```python
from build123d import *

# Parameters (mm, degrees)
BRACKET_BODY_DEPTH      = 35
EYE_END_ROUND_RADIUS    = 35
EYE_END_ROUND_LENGTH    = 20
FORK_GAP_CUT_DEPTH      = 106.59356041
FORK_GAP_CUT_DEPTH_BACK = 106.59356041
FORK_SLOT_CUT_DEPTH     = 15
EYE_BORE_30_REACH       = 110.858
EYE_BORE_SKETCH_R       = 15


with BuildPart() as part:
    # Bracket Profile Sketch → Bracket Body (new, symmetric)
    with BuildSketch(Plane.XY):
        with BuildLine():
            Line((40, -20), (0, -20))
            ThreePointArc((0, -20), (-20, 0), (0, 20))
            Line((0, 20), (40, 20))
            Line((40, 20), (40, 30))
            Line((40, 30), (-20, 30))
            Line((-20, 30), (-40, 10))
            Line((-40, 10), (-95, 10))
            Line((-95, 10), (-95, -10))
            Line((-95, -10), (-40, -10))
            Line((-40, -10), (-20, -30))
            Line((-20, -30), (40, -30))
            Line((40, -30), (40, -20))
        make_face()
    extrude(amount=BRACKET_BODY_DEPTH, both=True)

    # Eye End Round: full round fillet: the end face becomes a half cylinder, R = half its width
    eye_end_round_face = Plane((-95, 0, 0), x_dir=(0, -1, 0), z_dir=(-1, 0, 0))  # on the end face: x along it, z out of the body
    eye_end_round_slab = eye_end_round_face.offset(-EYE_END_ROUND_RADIUS / 2) * Box(EYE_END_ROUND_LENGTH, 2 * EYE_END_ROUND_RADIUS, EYE_END_ROUND_RADIUS, mode=Mode.PRIVATE)  # the body's end, R deep
    eye_end_round_round = Plane((-60, 0, 0), x_dir=(-1, 0, 0), z_dir=(0, -1, 0)) * Cylinder(EYE_END_ROUND_RADIUS, EYE_END_ROUND_LENGTH, mode=Mode.PRIVATE)  # its axis R under the face
    add(eye_end_round_slab - eye_end_round_round, mode=Mode.SUBTRACT)

    # Fork Gap Sketch → Fork Gap Cut (cut, two sides: drawn at the far end of the back side and taken through both)
    with BuildSketch(Plane(origin=(0, 0, 0), x_dir=(1, 0, 0), z_dir=(0, 1, 0)).offset(-FORK_GAP_CUT_DEPTH_BACK)):
        with BuildLine():
            Line((40, 10), (25, 10))
            ThreePointArc((25, 10), (15, 0), (25, -10))
            Line((25, -10), (40, -10))
            Line((40, -10), (40, 10))
        make_face()
    extrude(amount=FORK_GAP_CUT_DEPTH + FORK_GAP_CUT_DEPTH_BACK, mode=Mode.SUBTRACT)

    # Fork Slot Sketch → Fork Slot Cut (cut, symmetric)
    with BuildSketch(Plane.XY):
        Polygon((-40, 10), (-30, 10), (-30, 20), align=None)
    fork_slot_cut = extrude(amount=FORK_SLOT_CUT_DEPTH, both=True, mode=Mode.SUBTRACT)

    # Eye Bore Sketch → Eye Bore _30 (cut, up to next)
    with BuildSketch(Plane(origin=(0, 10, 0), x_dir=(1, 0, 0), z_dir=(0, 1, 0)), mode=Mode.PRIVATE) as eye_bore_30_sk1:
        with Locations(Location((-60, 0, 0), (0, 0, 180))):
            Circle(EYE_BORE_SKETCH_R)
    eye_bore_30_tool1 = extrude(eye_bore_30_sk1.sketch, amount=-EYE_BORE_30_REACH, mode=Mode.PRIVATE) & part.part
    add(eye_bore_30_tool1.solids().sort_by_distance((-60, 10, 0))[0], mode=Mode.SUBTRACT)

    # Fork Slot Mirror: Fork Slot Cut across plane
    add(fork_slot_cut.mirror(Plane.ZX), mode=Mode.SUBTRACT)


solid = part.part
```
CAD build for the part. Positions are in the model's coordinates, mm. A direction names the side the tool comes from. Coordinates: 2 decimals unless noted, no trailing zeros. Order: outer loops, then holes, each group sorted by start corner. A loop starts at its lowest first (then second) coordinate and runs counter-clockwise, first axis right, second up. Notation, with made-up numbers: (-9, -0.5) -> (34, -0.5) arc R30 ccw to (34, 36.5) -> close; hole circle Ø9 at (49.5, -4.75). An arc over 180 degrees is marked (long way). Use one line per item in the form item = value. Start each with the question number.
1) Band-saw the part on A-A on z = 0. Give the cut face in (x, y), then the cut area to 3 significant figures.
2) Band-saw the part on B-B on x = 6. Give the cut face in (y, z), then the cut area to 3 significant figures.
3) Band-saw the part on D-D on z = -23. Give the cut face in (x, y), then the cut area to 3 significant figures.
4) Band-saw the part on C-C on y = 0. Give the cut face in (x, z).
5) Drill centre lines: L1, parallel to Z at x = 27.5, y = 27; L2, parallel to Y at x = 11, z = -31; L3, parallel to Z at x = -60, y = -4.5. Where is each one in solid material? Low to high. Write a range as [from, to].
6) Drop flat-ended pins along their axis: pin 1 (6 mm diameter, centred on x = -52, z = -11, fed in from +Y); pin 2 (12 mm diameter, centred on y = 9, z = 7.5, fed in from -X); pin 3 (1 mm diameter, centred on y = -6, z = -10.5, fed in from +X). Give the stop position or say it passes through.
7) Pull direction Z, two halves, no side cores. Call faces 6 (the flat face through (40, 25, -22)), 7 (the flat face through (33, 25, -10)), 8 (the cylindrical face through (-94.99, -0.14, 0.77)), 9 (the flat face through (-22, 0, -35)): +Z half, -Z half, draft (parallel to the pull), parting line (faces both ways), or undercut.
8) Tool access for faces 1 (the flat face through (-33, 13, -15)), 2 (the flat face through (33, -25, -10)), 3 (the flat face through (11, -20, 0)), 4 (the flat face through (-33, -13, 15)), 5 (the flat face through (10, 30, 0)): list every direction of +Z, -Z, +X, -X, +Y, -Y with a clear straight run to the whole face (end or side of a thin tool).
Entries:
q1.outline = (-95, -10) -> (-75, -10) -> (-75, 10) -> (-95, 10) -> close; (-45, -10) -> (-30, -10) -> (-30, -20) -> (-20, -30) -> (15, -30) -> (15, -20) -> (0, -20) arc R20 cw to (0, 20) -> (15, 20) -> (15, 30) -> (-20, 30) -> (-30, 20) -> (-30, 10) -> (-45, 10) -> close
q1.area = 2,070 mm2
q2.outline = (-30, -35) -> (-20, -35) -> (-20, 35) -> (-30, 35) -> close; (20, -35) -> (30, -35) -> (30, 35) -> (20, 35) -> close
q2.area = 1,400 mm2
q3.outline = (-86.38, -10) -> (-40, -10) -> (-20, -30) -> (40, -30) -> (40, -20) -> (0, -20) arc R20 cw to (0, 20) -> (40, 20) -> (40, 30) -> (-20, 30) -> (-40, 10) -> (-86.38, 10) -> close
q3.area = 3,100 mm2
q4.outline = (-60, -35) -> (-20, -35) -> (-20, 35) -> (-60, 35) arc R35 ccw to start; hole circle Ø30 at (-60, 0)
q5.L1 = [-35, -10], [10, 35]
q5.L2 = [-30, -20], [20, 30]
q5.L3 = [-35, -15], [15, 35]
q6.pin_1 = 10
q6.pin_2 = -94.97
q6.pin_3 = -18.91
q7.face_6 = draft
q7.face_7 = undercut
q7.face_8 = parting line
q7.face_9 = -Z half
q8.face_1 = -X, +Y
q8.face_2 = +X, +Y, -Y
q8.face_3 = +Z, -Z, +X
q8.face_4 = -X, -Y
q8.face_5 = +Z, -Z, +X, -X, +Y
